Verification items for the finished model (mm, model axes). A direction names the side the tool comes from. Round coordinates to 2 decimals unless told otherwise and drop trailing zeros. Write each loop counter-clockwise with the first axis right and the second up, starting at its lowest first coordinate (ties: lowest second). Pieces come first, ordered by that corner, then holes. Notation, with made-up numbers: (-37, 65) - (-19, 65) arc R15 cw to (-19, 88) - close; hole circle Ø4 at (75.25, 74). An arc over 180 degrees is marked (long way). Write each question's results on one line, items separated by ' | '.
```python
from build123d import *

# Parameters (mm, degrees)
EXTRUDE_1_DEPTH    = 575
HOLE_WIZARD_M4_1_D = 3.3
HOLE_WIZARD_M6_1_D = 5
HOLE_WIZARD_M8_1_D = 6.8
HOLE_WIZARD_M6_2_D = 5


with BuildPart() as part:
    # 草图1 → 凸台-拉伸1 (new, symmetric)
    with BuildSketch(Plane.XY):
        Polygon((0, 0), (120, 0), (120, -75), (110, -75), (110, -10), (0, -10), align=None)
    extrude(amount=EXTRUDE_1_DEPTH, both=True)

    # M4 螺纹孔1 (through all)
    with Locations(Plane(origin=(0, 0, 0), x_dir=(1, 0, 0), z_dir=(0, 1, 0))):
        with Locations((5.2, 43.6), (21.1, 43.6), (5.2, 24.6), (21.1, 24.6), (5.2, -134.6), (21.1, -134.6), (5.2, -153.6), (21.1, -153.6), (5.2, -551.4), (21.1, -551.4), (5.2, -570.4), (21.1, -570.4), (5.2, 570.4), (21.1, 570.4), (21.1, 551.4), (5.2, 551.4)):
            Hole(HOLE_WIZARD_M4_1_D / 2)

    # M6 螺纹孔1 (through all)
    with Locations(Plane(origin=(0, 0, 0), x_dir=(1, 0, 0), z_dir=(0, 1, 0))):
        with Locations((20, 308.5), (50, 308.5), (20, -418.5), (50, -418.5)):
            Hole(HOLE_WIZARD_M6_1_D / 2)

    # M8 螺纹孔1 (through all)
    with Locations(Plane(origin=(0, 0, 0), x_dir=(1, 0, 0), z_dir=(0, 1, 0))):
        with Locations((25, 188.5), (60, 188.5), (95, 188.5), (95, 138.5), (60, 138.5), (25, 138.5), (25, -248.5), (60, -248.5), (95, -248.5), (95, -298.5), (60, -298.5), (25, -298.5)):
            Hole(HOLE_WIZARD_M8_1_D / 2)

    # M6 螺纹孔2 (through all)
    with Locations(Plane(origin=(120, 0, 0), x_dir=(0, 0, -1), z_dir=(1, 0, 0))):
        with Locations((-568.6, -49.6), (-537, -49.6), (-537, -68.6), (-568.6, -68.6), (-15.8, -49.6), (15.8, -49.6), (15.8, -68.6), (-15.8, -68.6), (537, -49.6), (568.6, -49.6), (568.6, -68.6), (537, -68.6)):
            Hole(HOLE_WIZARD_M6_2_D / 2)


solid = part.part
```
(1) Set-up check for faces 1 (the flat face through (78.1, -9.5, -575)), 2 (the flat face through (110, -43, 8)): record each of +Z, -Z, +X, -X, +Y, -Y from which the full face is reachable in a straight line by a thin tool's end or side.
Answer:
face 1: -Z, +X, -X, +Y, -Y | face 2: +Z, -Z, -X, -Y
(2) Go/stop test with flat-tipped pins: pin 1 Ø3 at (x, z) = (69.5, -68) entering from -Y; pin 2 Ø5.5 at (x, z) = (95, 298.5) entering from -Y; pin 3 Ø2 at (y, z) = (-63, 415) entering from -X. Record where each tip stops, or that it passes through.
Answer:
pin 1: y = -10 | pin 2: through | pin 3: x = 110
(3) Section check B-B (y = -30). Record the cut outline in (x, z).
Answer:
outline: (110, -575) - (120, -575) - (120, 575) - (110, 575) - close
(4) Thickness scan on L1, parallel to Z at x = 25, y = -4.5; L2, parallel to X at y = -2, z = 570; L3, parallel to Z at x = 49, y = -3.5. Record the ranges inside material, lowest first.
Answer:
L1: -575 to -191.9, -185.1 to -141.9, -135.1 to 245.1, 251.9 to 295.1, 301.9 to 575 | L2: 0 to 3.6, 6.8 to 19.5, 22.7 to 120 | L3: -575 to -310.79, -306.21 to 416.21, 420.79 to 575
(5) Section check A-A (z = 181). Record the cut outline in (x, y).
Answer:
outline: (0, -10) - (110, -10) - (110, -75) - (120, -75) - (120, 0) - (0, 0) - close
